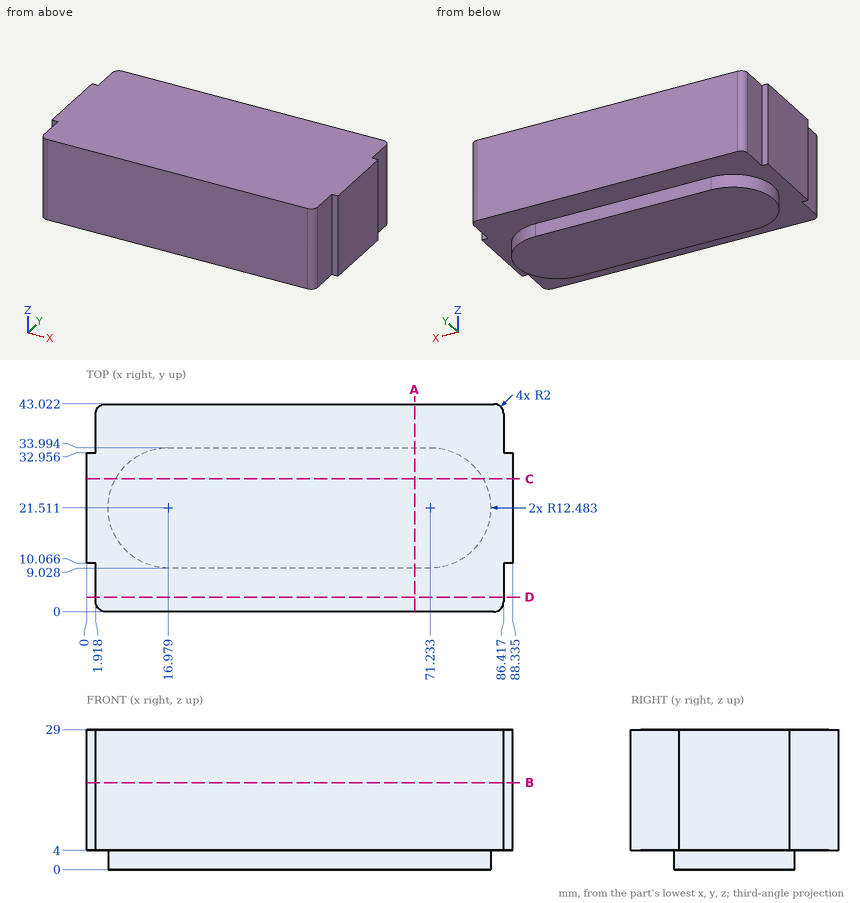
Job drawing, mm, ordinate dimensions from the low corner. One solid piece. Give positions to 0.01 mm unless a question says otherwise; leave off trailing zeros. Order: outer loops, then holes, each group sorted by start corner. A loop starts at its lowest first (then second) coordinate and runs counter-clockwise, first axis right, second up. Notation, with made-up numbers: (19.25, 13) - (29.25, 13) arc R32 ccw to (29.25, 39) - close; hole circle Ø2 at (53.25, -1). An arc over 180 degrees is marked (long way). Return JSON: item names as keys, results as strings.
1) Probe line 1 (Y direction, x = 49, z = 2.5); line 2 (X direction, y = 38, z = 9.5); line 3 (Z direction, x = 32, y = 8). List the from-to ranges inside material, lowest first. Write a range as from..to.
Geometry says:
{"line 1": "9.03..33.99", "line 2": "1.92..86.42", "line 3": "4..29"}
2) Cut at B-B, the plane z = 18. Give the cut face in (x, y) (1 decimal).
Geometry says:
{"outline": "(0, 10.1) - (1.9, 10.1) - (1.9, 2) arc R2 ccw to (3.9, 0) - (84.4, 0) arc R2 ccw to (86.4, 2) - (86.4, 10.1) - (88.3, 10.1) - (88.3, 33) - (86.4, 33) - (86.4, 41) arc R2 ccw to (84.4, 43) - (3.9, 43) arc R2 ccw to (1.9, 41) - (1.9, 33) - (0, 33) - close"}
3) Flat gauge pins, fed straight in: P1, Ø1.2, axis at x = 54.5, z = 1.5, coming from the -Y side; P2, Ø2, axis at x = 87, z = 22.5, coming from the -Y side; P3, Ø6.5, axis at y = 6.5, z = 11.5, coming from the +X side. Where does each tip first touch, or does it go through?
Geometry says:
{"P1": "y = 9.03", "P2": "y = 0.78", "P3": "x = 86.42"}
4) Cut at D-D, the plane y = 3. Give the cut face in (x, z).
Geometry says:
{"outline": "(1.92, 4) - (86.42, 4) - (86.42, 29) - (1.92, 29) - close"}
5) Cut at A-A, the plane x = 68. Give the cut face in (y, z).
Geometry says:
{"outline": "(0, 4) - (9.03, 4) - (9.03, 0) - (33.99, 0) - (33.99, 4) - (43.02, 4) - (43.02, 29) - (0, 29) - close"}
6) Cut at C-C, the plane y = 27.5. Give the cut face in (x, z) (1 decimal), plus the area to 3 significant figures.
Geometry says:
{"outline": "(0, 4) - (6, 4) - (6, 0) - (82.2, 0) - (82.2, 4) - (88.3, 4) - (88.3, 29) - (0, 29) - close", "area": "2,510 mm²"}
